Read the model definition and answer for the solid it produces. Units are mm, in the model's axes. Give positions to 0.01 mm unless a question says otherwise; leave off trailing zeros. Write each loop counter-clockwise with the first axis right and the second up, starting at its lowest first coordinate (ties: lowest second). Pieces come first, ordered by that corner, then holes. Notation, with made-up numbers: (53.5, 35) - (110.5, 35) arc R31 cw to (110.5, 70) - close; hole circle Ø2 at (58.25, 5.25). An arc over 180 degrees is marked (long way). Answer as CSV lines item,"result".
```python
from build123d import *

# Parameters (mm, degrees)
BOSS_EXTRUDE1_DEPTH = 2660


with BuildPart() as part:
    # Sketch1 → Boss-Extrude1 (new body)
    with BuildSketch(Plane.XY):
        with BuildLine():
            Line((-70.999999998, 146), (-70.999999998, 70))
            ThreePointArc((-70.999999998, 70), (-72.757359311, 65.757359313), (-76.999999998, 64))
            Line((-76.999999998, 64), (-120.999999998, 64))
            Line((-120.999999998, 64), (-120.999999998, 58))
            Line((-120.999999998, 58), (-76.999999998, 58))
            ThreePointArc((-76.999999998, 58), (-68.514718624, 61.514718626), (-64.999999998, 70))
            Line((-64.999999998, 70), (-64.999999998, 146))
            ThreePointArc((-64.999999998, 146), (-63.242640685, 150.242640687), (-58.999999998, 152))
            Line((-58.999999998, 152), (91, 152))
            ThreePointArc((91, 152), (95.242640687, 150.242640687), (97, 146))
            Line((97, 146), (97, 76))
            ThreePointArc((97, 76), (95.242640687, 71.757359313), (91, 70))
            Line((91, 70), (56, 70))
            ThreePointArc((56, 70), (47.514718626, 66.485281374), (44, 58))
            Line((44, 58), (44, 12))
            ThreePointArc((44, 12), (42.242640687, 7.757359313), (38, 6))
            Line((38, 6), (0, 6))
            Line((0, 6), (0, 0))
            Line((0, 0), (38, 0))
            ThreePointArc((38, 0), (46.485281374, 3.514718626), (50, 12))
            Line((50, 12), (50, 58))
            ThreePointArc((50, 58), (51.757359313, 62.242640687), (56, 64))
            Line((56, 64), (91, 64))
            ThreePointArc((91, 64), (99.485281374, 67.514718626), (103, 76))
            Line((103, 76), (103, 146))
            ThreePointArc((103, 146), (99.485281374, 154.485281374), (91, 158))
            Line((91, 158), (-58.999999998, 158))
            ThreePointArc((-58.999999998, 158), (-67.485281372, 154.485281374), (-70.999999998, 146))
        make_face()
    extrude(amount=BOSS_EXTRUDE1_DEPTH)


solid = part.part
```
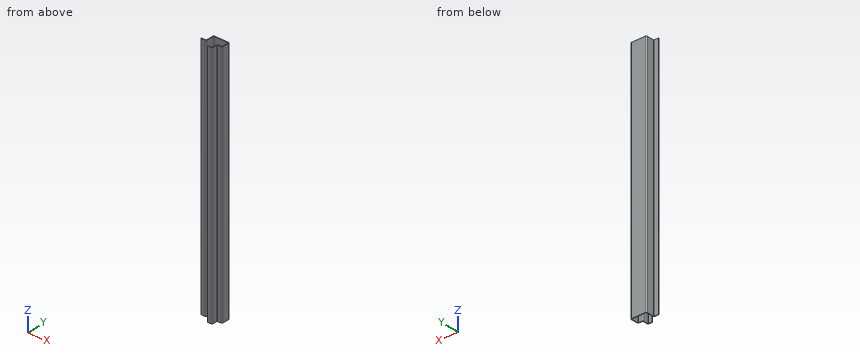
(1) Each of these flat-tipped pins is pushed along its axis until it touches: P1, Ø3, axis at y = 74, z = 293.5, coming from the -X side; P2, Ø3, axis at y = 68, z = 315, coming from the -X side; P3, Ø23, axis at y = 25, z = 1147, coming from the +X side. Where does it stop, or does it pass through?
Worked out:
P1,"stops at x = -71"
P2,"stops at x = -72.13"
P3,"stops at x = 50"
(2) A cutting plane is placed at B-B (z = 1922). Write down the section's boundary in (x, y), and give its area (3 significant figures).
Worked out:
outline,"(-121, 58) - (-77, 58) arc R12 ccw to (-65, 70) - (-65, 146) arc R6 cw to (-59, 152) - (91, 152) arc R6 cw to (97, 146) - (97, 76) arc R6 cw to (91, 70) - (56, 70) arc R12 ccw to (44, 58) - (44, 12) arc R6 cw to (38, 6) - (0, 6) - (0, 0) - (38, 0) arc R12 ccw to (50, 12) - (50, 58) arc R6 cw to (56, 64) - (91, 64) arc R12 ccw to (103, 76) - (103, 146) arc R12 ccw to (91, 158) - (-59, 158) arc R12 ccw to (-71, 146) - (-71, 70) arc R6 cw to (-77, 64) - (-121, 64) - close"
area,"3,260 mm^2"
(3) Find the intervals of material crossed by L1, parallel to X at y = 141.5, z = 1375.5; L2, parallel to Y at x = 32, z = 1955; L3, parallel to X at y = 59.5, z = 346.5, in increasing order.
Worked out:
L1,"x = -71 to -65, 97 to 103"
L2,"y = 0 to 6, 152 to 158"
L3,"x = -121 to -71.19, 44.09 to 50.19"
(4) A cutting plane is placed at C-C (x = -22.5). Write down the section's boundary in (y, z), and give its area (3 significant figures).
Worked out:
outline,"(152, 0) - (158, 0) - (158, 2660) - (152, 2660) - close"
area,"16,000 mm^2"
(5) A cutting plane is placed at A-A (y = 106.5). Write down the section's boundary in (x, z), and give its area (3 significant figures).
Worked out:
outline,"(-71, 0) - (-65, 0) - (-65, 2660) - (-71, 2660) - close; (97, 0) - (103, 0) - (103, 2660) - (97, 2660) - close"
area,"31,900 mm^2"
